Here's how the part is built. I have some questions about the finished solid (model axes, mm). Face numbers are marked on the shaded views. A direction names the side the tool comes from. Give positions to 0.01 mm unless a question says otherwise; leave off trailing zeros. Order: outer loops, then holes, each group sorted by start corner. A loop starts at its lowest first (then second) coordinate and runs counter-clockwise, first axis right, second up. Notation, with made-up numbers: M 36.5,16.5 L 88.5,16.5 A16 cw 88.5,45.5 Z; hole C 54.25,-23 d9. An arc over 180 degrees is marked long. Use one line per item in the form item = value.
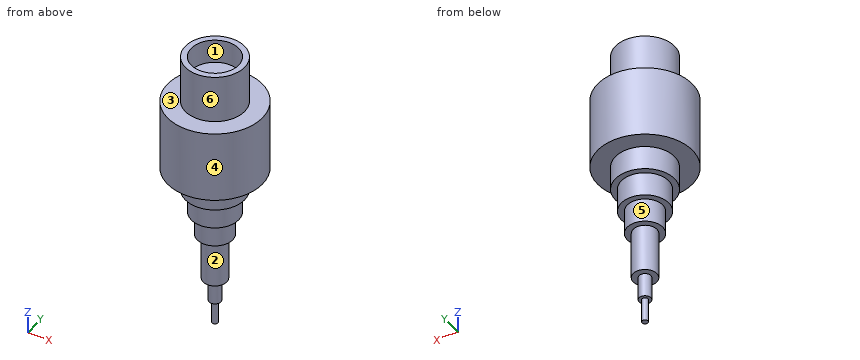
from build123d import *

# Parameters (mm, degrees)
COLLAR_PROFILE_80_R     = 40
COLLAR_80_DEPTH         = 60
SPIGOT_SKETCH_50_R      = 25
SPIGOT_50_DEPTH         = 40
SPIGOT_BORE_SKETCH_40_R = 20
SPIGOT_BORE_40_DEPTH    = 20
PIN_START               = 20
PIN_STEP_1_SKETCH_50_R  = 25
PIN_STEP_1_50_DEPTH     = 20
PIN_STEP_2_SKETCH_40_R  = 20
PIN_STEP_2_40_DEPTH     = 20
PIN_STEP_3_SKETCH_30_R  = 15
PIN_STEP_3_30_DEPTH     = 20
PIN_STEP_4_SKETCH_20_R  = 10
PIN_STEP_4_20_DEPTH     = 20
PIN_STEP_5_SKETCH_20_R  = 10
PIN_STEP_5_20_DEPTH     = 20
PIN_STEP_6_SKETCH_10_R  = 5
PIN_STEP_6_10_DEPTH     = 20
PIN_TIP_SKETCH_5_R      = 2.5
PIN_TIP_5_DEPTH         = 20


with BuildPart() as part:
    # Collar Profile Ø80 → Collar Ø80 (new body)
    with BuildSketch(Plane.XY):
        Circle(COLLAR_PROFILE_80_R)
    extrude(amount=COLLAR_80_DEPTH)

    # Spigot Sketch Ø50 → Spigot Ø50 (add)
    with BuildSketch(Plane.XY.offset(60)):
        Circle(SPIGOT_SKETCH_50_R)
    extrude(amount=SPIGOT_50_DEPTH)

    # Spigot Bore Sketch Ø40 → Spigot Bore Ø40 (cut)
    with BuildSketch(Plane.XY.offset(100)):
        Circle(SPIGOT_BORE_SKETCH_40_R)
    extrude(amount=-SPIGOT_BORE_40_DEPTH, mode=Mode.SUBTRACT)

    # Pin Step 1 Sketch Ø50 → Pin Step 1 Ø50 (add)
    with BuildSketch(Plane(origin=(0, 0, 0), x_dir=(-1, 0, 0), z_dir=(0, 0, -1)).offset(PIN_START)):
        with Locations(Location((0, 0, 0), (0, 0, 180))):
            Circle(PIN_STEP_1_SKETCH_50_R)
    extrude(amount=-PIN_STEP_1_50_DEPTH)

    # Pin Step 2 Sketch Ø40 → Pin Step 2 Ø40 (add)
    with BuildSketch(Plane(origin=(0, 0, -20), x_dir=(-1, 0, 0), z_dir=(0, 0, -1))):
        with Locations(Location((0, 0, 0), (0, 0, 180))):
            Circle(PIN_STEP_2_SKETCH_40_R)
    extrude(amount=PIN_STEP_2_40_DEPTH)

    # Pin Step 3 Sketch Ø30 → Pin Step 3 Ø30 (add)
    with BuildSketch(Plane(origin=(0, 0, -40), x_dir=(-1, 0, 0), z_dir=(0, 0, -1))):
        Circle(PIN_STEP_3_SKETCH_30_R)
    extrude(amount=PIN_STEP_3_30_DEPTH)

    # Pin Step 4 Sketch Ø20 → Pin Step 4 Ø20 (add)
    with BuildSketch(Plane(origin=(0, 0, -60), x_dir=(-1, 0, 0), z_dir=(0, 0, -1))):
        Circle(PIN_STEP_4_SKETCH_20_R)
    extrude(amount=PIN_STEP_4_20_DEPTH)

    # Pin Step 5 Sketch Ø20 → Pin Step 5 Ø20 (add)
    with BuildSketch(Plane(origin=(0, 0, -80), x_dir=(-1, 0, 0), z_dir=(0, 0, -1))):
        Circle(PIN_STEP_5_SKETCH_20_R)
    extrude(amount=PIN_STEP_5_20_DEPTH)

    # Pin Step 6 Sketch Ø10 → Pin Step 6 Ø10 (add)
    with BuildSketch(Plane(origin=(0, 0, -100), x_dir=(-1, 0, 0), z_dir=(0, 0, -1))):
        Circle(PIN_STEP_6_SKETCH_10_R)
    extrude(amount=PIN_STEP_6_10_DEPTH)

    # Pin Tip Sketch Ø5 → Pin Tip Ø5 (add)
    with BuildSketch(Plane(origin=(0, 0, -120), x_dir=(-1, 0, 0), z_dir=(0, 0, -1))):
        Circle(PIN_TIP_SKETCH_5_R)
    extrude(amount=PIN_TIP_5_DEPTH)


solid = part.part
Q1. Thinking about a two-plate mould opening in Y: for the marked faces 1, 2 and 3, which applies, +Y half, -Y half, draft (parallel to the pull), parting line (faces both ways), or undercut?
Found:
face_1 = undercut
face_2 = parting line
face_3 = draft
Q2. I need wall thicknesses on L1, parallel to Y at x = 0, z = 92; L2, parallel to Z at x = -29.5, y = -21; L3, parallel to Z at x = -15, y = -5.5. Which ranges of each line are inside material? Lowest first, please.
Found:
L1 = -25 to -20, 20 to 25
L2 = 0 to 60
L3 = -40 to 80
Q3. I want a section at A-A on z = 33.5. Write out the boundary of the cut face in (x, y).
Found:
outline = C 0,0 d80
Q4. On a 3-axis mill with a long thin cutter (end or side, diameter ignored), from which of +Z, -Z, +X, -X, +Y, -Y can I reach the whole of each face in a straight line? I mean the marked faces 4, 5 and 6. Say none if no direction works.
Found:
face_4 = +Z, -Z
face_5 = -Z
face_6 = +Z
Q5. I'm going to push flat-ended pins straight in: pin 1 Ø1 at (y, z) = (-14.5, -9) entering from +X; pin 2 Ø12 at (y, z) = (-13.5, -55.5) entering from +X; pin 3 Ø10 at (x, y) = (4.5, -18) entering from -Z; pin 4 Ø3 at (x, y) = (-2, -2) entering from -Z. Where does each tip first touch, or does it pass through?
Found:
pin_1 = 20.71
pin_2 = 12.99
pin_3 = -60
pin_4 = -140
Q6. I want a section at D-D on z = -74. Write out the boundary of the cut face in (x, y).
Found:
outline = C 0,0 d20
Q7. I want a section at B-B on x = 7.5. Write out the boundary of the cut face in (y, z), then the cut area to 3 significant figures.
Found:
outline = M -39.29,0 L -23.85,0 L -23.85,-20 L -18.54,-20 L -18.54,-40 L -12.99,-40 L -12.99,-60 L -6.61,-60 L -6.61,-100 L 6.61,-100 L 6.61,-60 L 12.99,-60 L 12.99,-40 L 18.54,-40 L 18.54,-20 L 23.85,-20 L 23.85,0 L 39.29,0 L 39.29,60 L 23.85,60 L 23.85,100 L 18.54,100 L 18.54,80 L -18.54,80 L -18.54,100 L -23.85,100 L -23.85,60 L -39.29,60 Z
area = 8,630 mm²
Q8. I want a section at C-C on y = -31. Write out the boundary of the cut face in (x, z), then the cut area to 3 significant figures.
Found:
outline = M -25.28,0 L 25.28,0 L 25.28,60 L -25.28,60 Z
area = 3,030 mm²
